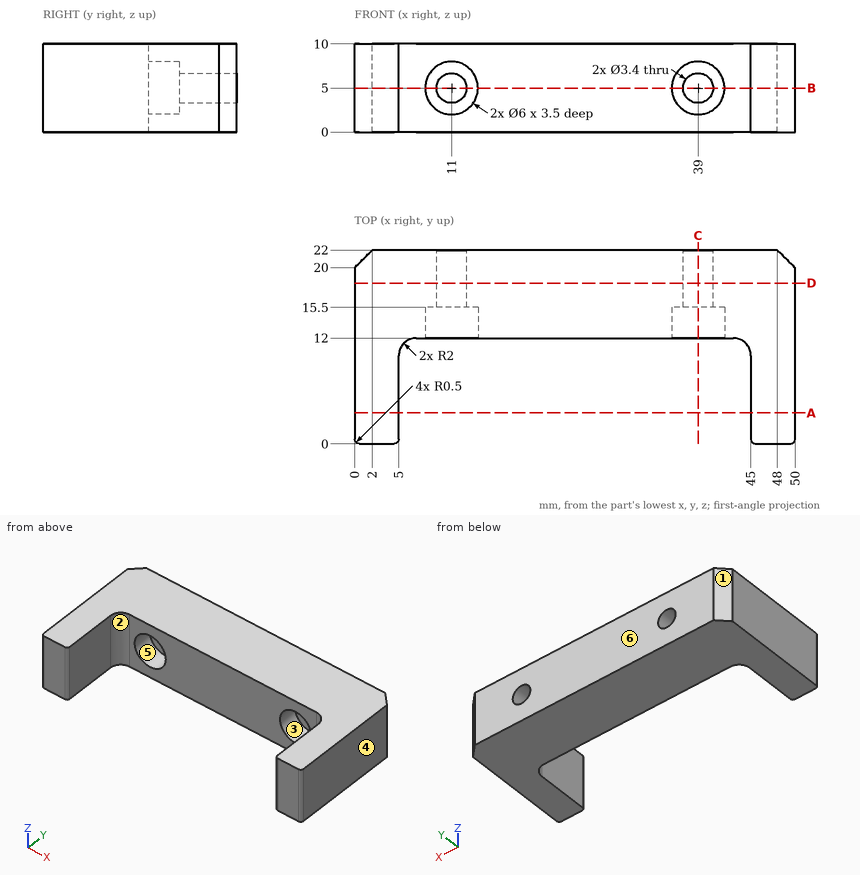
The drawing under review shows one solid part. Ordinate dimensions are in mm from its lowest x, y, z. A direction names the side the tool comes from. Give positions to 0.01 mm unless a question says otherwise; leave off trailing zeros. Loops run counter-clockwise (first coordinate to the right, second up) from the corner with the lowest first, then second, coordinate; pieces in that order, holes last. Notation, with made-up numbers: M -1,6.5 L 21,6.5 A23 ccw 21,19.5 Z; hole C 50,20.5 d1. An arc over 180 degrees is marked long. Return JSON: item names as keys, results as strings. Group by question number.
Item 1: We need section B-B (z = 5). Give the number of separate pieces and of enclosed holes in the cut face, and give its area (3 significant figures).
Item 2: Tool access review of the marked faces 1, 2 and 3: name each direction out of +Z, -Z, +X, -X, +Y, -Y from which nothing blocks a thin tool from reaching the whole face with its end or side.
Item 3: We need section D-D (y = 18.25). Give the boundary of the cut face in (x, z), and give its area (3 significant figures).
Item 4: We need section C-C (x = 39). Give the boundary of the cut face in (y, z).
Item 5: For probe 1 along Z at (x, y) = (39, 12.9); probe 2 along Z at (x, y) = (39, 18); probe 3 along X at (y, z) = (20.25, 3.5), list the stretches that pass through material, from the lowest coordinate up.
Item 6: Mouldability with a two-part tool opening along X and no side actions: class the marked faces 4, 5 and 6 as released by +X, released by -X, zero draft, split by the parting line, or undercut.
Item 7: Insertion check: pin 1 Ø2.5 at (x, z) = (39, 5) entering from -Y (3 decimals); pin 2 Ø10 at (x, y) = (28.5, 9.5) entering from -Z; pin 3 Ø5 at (x, z) = (10, 5.5) entering from -Y; pin 4 Ø3.5 at (x, z) = (11, 5) entering from -Y. Each pin has a flat end and moves straight along its axis. Give the tip position at first contact, or say it passes through.
Item 8: We need section A-A (y = 3.5). Give the boundary of the cut face in (x, z).
Output:
{
 "1": {"separate pieces": "3", "enclosed holes": "0", "area": "531 mm^2"},
 "2": {"face 1": "+Z, -Z, -X, +Y", "face 2": "+Z, -Z, -Y", "face 3": "-Y"},
 "3": {"outline": "M 0,0 L 50,0 L 50,10 L 0,10 Z; hole C 11,5 d3.4; hole C 39,5 d3.4", "area": "482 mm^2"},
 "4": {"outline": "M 12,0 L 22,0 L 22,3.3 L 15.5,3.3 L 15.5,2 L 12,2 Z; M 12,8 L 15.5,8 L 15.5,6.7 L 22,6.7 L 22,10 L 12,10 Z"},
 "5": {"probe 1": "z = 0 to 2, 8 to 10", "probe 2": "z = 0 to 3.3, 6.7 to 10", "probe 3": "x = 0.25 to 10.2, 11.8 to 38.2, 39.8 to 49.75"},
 "6": {"face 4": "released by +X", "face 5": "undercut", "face 6": "zero draft"},
 "7": {"pin 1": "passes through", "pin 2": "stops at z = 0", "pin 3": "stops at y = 12", "pin 4": "stops at y = 15.5"},
 "8": {"outline": "M 0,0 L 5,0 L 5,10 L 0,10 Z; M 45,0 L 50,0 L 50,10 L 45,10 Z"}
}
